Design review of the part built by this model. Coordinates are the model's own, in mm. A direction names the side the tool comes from. Coordinates: 2 decimals unless noted, no trailing zeros. Write each loop counter-clockwise with the first axis right and the second up, starting at its lowest first coordinate (ties: lowest second). Pieces come first, ordered by that corner, then holes. Notation, with made-up numbers: M 17.5,18 L 64.5,18 A20 ccw 64.5,46 Z; hole C 67,7 d3. An arc over 180 degrees is marked long. Write item = value, one per line.
```python
from build123d import *

# Parameters (mm, degrees)
SKETCH1_W                                         = 225
SKETCH1_H                                         = 156
EXTRUDE1_DEPTH                                    = 4
M5_SOCKET_HEAD_CAP_SCREW_COUNTERBORE1_D           = 5.5
M5_SOCKET_HEAD_CAP_SCREW_COUNTERBORE1_CBORE_D     = 10
M5_SOCKET_HEAD_CAP_SCREW_COUNTERBORE1_CBORE_DEPTH = 6
M4_TAPPED_HOLE1_D                                 = 3.3
M4_TAPPED_HOLE2_D                                 = 3.3


with BuildPart() as part:
    # Sketch1 → Extrude1 (new, symmetric)
    with BuildSketch(Plane(origin=(0, 0, 0), x_dir=(1, 0, 0), z_dir=(0, 1, 0))):
        Rectangle(SKETCH1_W, SKETCH1_H)
    extrude(amount=EXTRUDE1_DEPTH, both=True)

    # M5 Socket Head Cap Screw Counterbore1 (through all)
    with Locations(Plane(origin=(105, 4, 70), x_dir=(0, 0, 1), z_dir=(0, 1, 0))):
        with Locations((0, 0), (-70, 0), (-140, 0)):
            m5_socket_head_cap_screw_counterbore1 = CounterBoreHole(M5_SOCKET_HEAD_CAP_SCREW_COUNTERBORE1_D / 2, M5_SOCKET_HEAD_CAP_SCREW_COUNTERBORE1_CBORE_D / 2, M5_SOCKET_HEAD_CAP_SCREW_COUNTERBORE1_CBORE_DEPTH)

    # Mirror1: M5 Socket Head Cap Screw Counterbore1 across plane
    add(m5_socket_head_cap_screw_counterbore1.mirror(Plane(origin=(0, 0, 0), x_dir=(0, 0, 1), z_dir=(1, 0, 0))), mode=Mode.SUBTRACT)

    # M4 Tapped Hole1 (through all)
    with Locations(Plane(origin=(101.5, 4, 25), x_dir=(0, 0, 1), z_dir=(0, 1, 0))):
        with Locations((0, 0), (-50, 0)):
            m4_tapped_hole1 = Hole(M4_TAPPED_HOLE1_D / 2)

    # M4 Tapped Hole2 (through all)
    with Locations(Plane(origin=(-33.5, 4, 70.5), x_dir=(0, 0, 1), z_dir=(0, 1, 0))):
        with Locations((0, 0), (0, 80)):
            m4_tapped_hole2 = Hole(M4_TAPPED_HOLE2_D / 2)

    # Mirror2: M4 Tapped Hole1 across plane
    add(m4_tapped_hole1.mirror(Plane(origin=(0, 0, 0), x_dir=(0, 0, 1), z_dir=(1, 0, 0))), mode=Mode.SUBTRACT)

    # Mirror3: M4 Tapped Hole2 across plane
    add(m4_tapped_hole2.mirror(Plane.XY), mode=Mode.SUBTRACT)


solid = part.part
```
Q1. Consider section A-A, the plane y = 2. State how many separate pieces and enclosed holes the cut face has, and give its area (3 significant figures).
Check result:
separate_pieces = 1
enclosed_holes = 14
area = 34,600 mm²
Q2. Machinability: for faces 4 (the flat face through (-2, -4, -1)), 5 (the flat face through (102.8, -2, 2.2)), which of the approach directions +Z, -Z, +X, -X, +Y, -Y give a long, thin tool a straight path to every point of the face, cutting with its end or side? Answer none if there is none.
Check result:
face_4 = +Z, -Z, +X, -X, -Y
face_5 = +Y
Q3. The part is to be moulded in two halves that separate along X. For faces 1 (the cylindrical face through (103.085, 1.042, -65.381)), 2 (the flat face through (112.5, 0, 1)), 3 (the flat face through (-2, 0, 78)), say which applies: +X half, -X half, draft (parallel to the pull), parting line (faces both ways), or undercut.
Check result:
face_1 = undercut
face_2 = +X half
face_3 = draft
Q4. For P1, Ø5, axis at x = 106.5, z = 71.5, coming from the +Y side; P2, Ø11.5, axis at x = 105, z = 70, coming from the -Y side, all flat-tipped, find the tip position at first contact; note any pin that passes through.
Check result:
P1 = -2
P2 = -4
Q5. Consider section B-B, the plane z = 0. State the section outline as (x, y) points.
Check result:
outline = M -112.5,-4 L -107.75,-4 L -107.75,-2 L -110,-2 L -110,4 L -112.5,4 Z; M -102.25,-4 L 102.25,-4 L 102.25,-2 L 100,-2 L 100,4 L -100,4 L -100,-2 L -102.25,-2 Z; M 107.75,-4 L 112.5,-4 L 112.5,4 L 110,4 L 110,-2 L 107.75,-2 Z
Q6. Wall thickness on line 1 (Z direction, x = -105, y = -3.4); line 2 (X direction, y = 2, z = -25); line 3 (Z direction, x = -103, y = -3.5): over which ranges is each line inside the solid? List them lowest first.
Check result:
line_1 = -78 to -72.75, -67.25 to -2.75, 2.75 to 67.25, 72.75 to 78
line_2 = -112.5 to -103.15, -99.85 to 99.85, 103.15 to 112.5
line_3 = -78 to -71.89, -68.11 to -25.69, -24.31 to -1.89, 1.89 to 24.31, 25.69 to 68.11, 71.89 to 78
